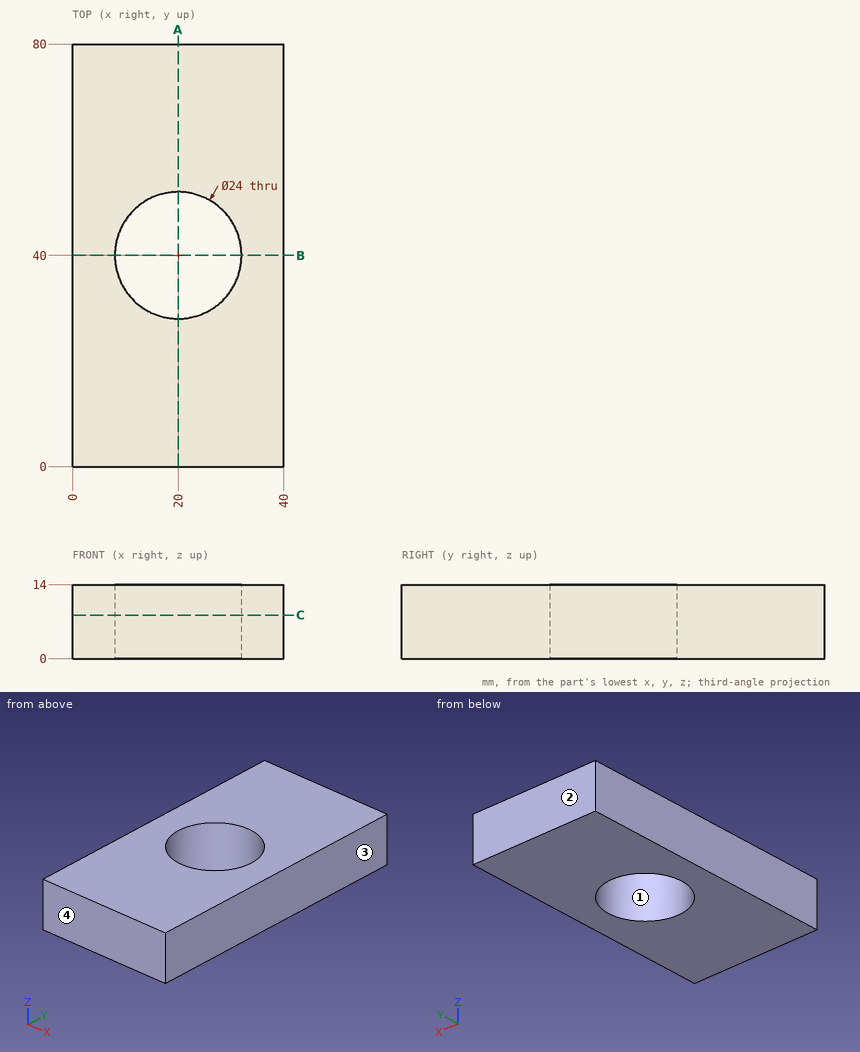
Geometry check sheet. Reference: drawing and pictorial views, mm from the part's lowest x, y, z. Give positions to 0.01 mm unless a question says otherwise; leave off trailing zeros. Order: outer loops, then holes, each group sorted by start corner. A loop starts at its lowest first (then second) coordinate and runs counter-clockwise, first axis right, second up. Notation, with made-up numbers: M 39,78 L 63,78 A28 cw 63,96 Z; hole C -36.75,-32.5 d6. An arc over 180 degrees is marked long. Answer in a Markdown table with one row per item. Add a question column.
Q1. Gauge pin test, flat end, axial feed: pin 1 Ø3 at (x, y) = (14.5, 15) entering from -Z. Record the tip position at first contact, or that the pin passes through.
Q2. Thickness scan on L1, parallel to Y at x = 20, z = 4; L2, parallel to X at y = 40.5, z = 1.5; L3, parallel to Y at x = 9, z = 8.75. Record the ranges inside material, lowest first.
Q3. Release check for a two-part mould opening along Y. For the marked faces 1, 2, 3 and 4 record: released by +Y, released by -Y, zero draft, split by the parting line, or undercut.
Q4. Sectioned sample at B-B, the plane y = 40. Record the boundary of the cut face in (x, z), and give its area (3 significant figures).
Q5. Sectioned sample at C-C, the plane z = 8.25. Record the boundary of the cut face in (x, y), and give its area (3 significant figures).
Q6. Sectioned sample at A-A, the plane x = 20. Record the boundary of the cut face in (y, z).
Verdict:
| question | item | result |
|---|---|---|
| 1 | pin 1 | z = 0 |
| 2 | L1 | 0 to 28, 52 to 80 |
| 2 | L2 | 0 to 8.01, 31.99 to 40 |
| 2 | L3 | 0 to 35.2, 44.8 to 80 |
| 3 | face 1 | undercut |
| 3 | face 2 | released by +Y |
| 3 | face 3 | zero draft |
| 3 | face 4 | released by -Y |
| 4 | outline | M 0,0 L 8,0 L 8,14 L 0,14 Z; M 32,0 L 40,0 L 40,14 L 32,14 Z |
| 4 | area | 224 mm² |
| 5 | outline | M 0,0 L 40,0 L 40,80 L 0,80 Z; hole C 20,40 d24 |
| 5 | area | 2,750 mm² |
| 6 | outline | M 0,0 L 28,0 L 28,14 L 0,14 Z; M 52,0 L 80,0 L 80,14 L 52,14 Z |
